Design review of the part built by this model. Coordinates are the model's own, in mm. Face numbers are marked on the shaded views. A direction names the side the tool comes from. Round coordinates to 2 decimals unless told otherwise and drop trailing zeros. Write each loop counter-clockwise with the first axis right and the second up, starting at its lowest first coordinate (ties: lowest second). Pieces come first, ordered by that corner, then holes.
from build123d import *

# Parameters (mm, degrees)
BOSS_EXTRUDE1_DEPTH   = 7.5
CUT_EXTRUDE1_REACH    = 84.706
SKETCH2_R             = 3.4
SKETCH3_R             = 14.05
SKETCH3_R_2           = 10.05
CUT_EXTRUDE2_DEPTH    = 15
FILLET1_R             = 5
M5_TAPPED_HOLE1_D     = 4.2
BODY_MOVE_COPY1_ANGLE = 180


with BuildPart() as part:
    # Sketch1 → Boss-Extrude1 (new, symmetric)
    with BuildSketch(Plane.XY):
        Polygon((40, 0), (-40, 0), (-40, 10), (-25, 10), (-25, 25), (-40, 25), (-40, 72), (40, 72), (40, 25), (25, 25), (25, 10), (40, 10), align=None)
    extrude(amount=BOSS_EXTRUDE1_DEPTH, both=True)

    # Sketch2 → Cut-Extrude1 (cut, up to next)
    with BuildSketch(Plane.XZ, mode=Mode.PRIVATE) as cut_extrude1_sk1:
        with Locations(Location((-35, 0, 0), (0, 0, 270))):
            Circle(SKETCH2_R)
    cut_extrude1_tool1 = extrude(cut_extrude1_sk1.sketch, amount=-CUT_EXTRUDE1_REACH, mode=Mode.PRIVATE) & part.part
    # Sketch2 → Cut-Extrude1 (cut, up to next)
    with BuildSketch(Plane.XZ, mode=Mode.PRIVATE) as cut_extrude1_sk2:
        with Locations(Location((35, 0, 0), (0, 0, 270))):
            Circle(SKETCH2_R)
    cut_extrude1_tool2 = extrude(cut_extrude1_sk2.sketch, amount=-CUT_EXTRUDE1_REACH, mode=Mode.PRIVATE) & part.part
    add(cut_extrude1_tool1.solids().sort_by_distance((-35, 0, 0))[0], mode=Mode.SUBTRACT)
    add(cut_extrude1_tool2.solids().sort_by_distance((35, 0, 0))[0], mode=Mode.SUBTRACT)

    # Sketch3 → Cut-Extrude2 (cut)
    with BuildSketch(Plane.XY.offset(7.5)):
        with Locations((-20, 52)):
            Circle(SKETCH3_R)
        with Locations((20, 52)):
            Circle(SKETCH3_R_2)
    extrude(amount=-CUT_EXTRUDE2_DEPTH, mode=Mode.SUBTRACT)

    # Fillet1
    fillet1_edges = [part.edges().sort_by_distance(p)[0] for p in [
        (-25, 10, 0),
        (-25, 25, 0),
        (-40, 25, 0),
        (-40, 72, 0),
        (40, 72, 0),
        (40, 25, 0),
        (25, 25, 0),
        (25, 10, 0),
    ]]
    fillet(fillet1_edges, radius=FILLET1_R)

    # M5 Tapped Hole1 (through all)
    with Locations(Plane(origin=(0, 0, -7.5), x_dir=(-1, 0, 0), z_dir=(0, 0, -1))):
        with Locations((33.435028843, 38.564971157), (6.564971157, 38.564971157), (6.564971157, 65.435028843), (33.435028843, 65.435028843)):
            Hole(M5_TAPPED_HOLE1_D / 2)


with BuildPart() as part_1:
    # Body-Move/Copy1: moved
    add(part.part.rotate(Axis((0, 30, 0), (0, 0, 1)), BODY_MOVE_COPY1_ANGLE))


solid = part_1.part
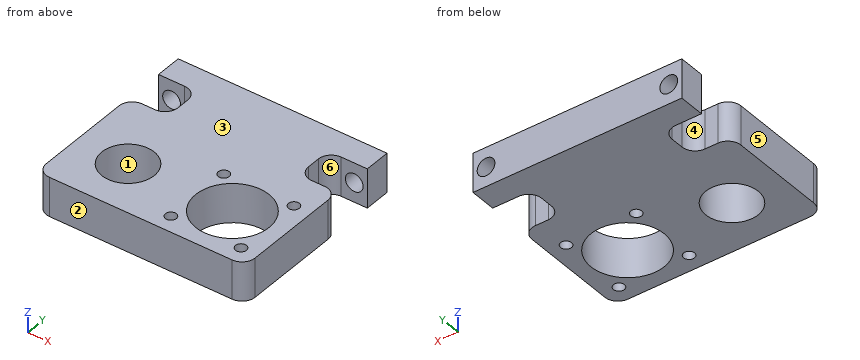
1) For line 1 along X through (y, z) = (8.5, -6.25); line 2 along Y through (x, z) = (20, -2.25); line 3 along Y through (x, z) = (-31.5, 6), list the stretches that pass through material, from the lowest coordinate up.
2) For the marked faces 4, 5 and 6, list the 3-axis set-ups (+Z, -Z, +X, -X, +Y, -Y) from which the entire face can be reached by the end or side of a thin tool; tool diameter is ignored.
3) The part is to be moulded in two halves that separate along Y. For the marked faces 1, 2 and 3, say which applies: pulls with the +Y half, pulls with the -Y half, needs draft (parallel to the pull), parting line crosses it, or undercut.
4) Add section C-C on z = -1.25. Count the separate pieces of the cut face and the enclosed holes in it, and give its area (3 significant figures).
5) Add section D-D on x = 28. State the section outline as (y, z) points, and give its area (3 significant figures).
6) For P1, Ø6, axis at x = -35, z = 0, coming from the +Y side; P2, Ø5.5, axis at y = 43, z = 0.5, coming from the -X side; P3, Ø1, axis at y = 37.5, z = 1.5, coming from the -X side, all flat-tipped, find the tip position at first contact; note any pin that passes through.
7) Add section A-A on x = -20. State the section outline as (y, z) points, and give its area (4 significant figures).
8) Add section B-B on y = 13. State the section outline as (x, z) points, and give its area (3 significant figures).
Computed:
1. line 1: x = -40 to -30.04, -9.96 to 5.96, 34.04 to 40
1. line 2: y = -12 to -6.05, 22.05 to 60
1. line 3: y = -12 to 35, 50 to 60
2. face 4: +Z, -Z, -X
2. face 5: +Z, -Z, -X, +Y, -Y
2. face 6: +Z, -Z, +X
3. face 1: undercut
3. face 2: pulls with the -Y half
3. face 3: needs draft
4. separate pieces: 3
4. enclosed holes: 6
4. area: 4,190 mm2
5. outline: (-12, -7.5) - (-3.55, -7.5) - (-3.55, 7.5) - (-12, 7.5) - close; (19.55, -7.5) - (35.42, -7.5) - (35.42, 7.5) - (19.55, 7.5) - close; (49.58, -7.5) - (60, -7.5) - (60, 7.5) - (49.58, 7.5) - close
5. area: 521 mm2
6. P1: stops at y = 35
6. P2: stops at x = -25.06
6. P3: stops at x = -26
7. outline: (-12, -7.5) - (-2.05, -7.5) - (-2.05, 7.5) - (-12, 7.5) - close; (18.05, -7.5) - (60, -7.5) - (60, 7.5) - (18.05, 7.5) - close
7. area: 778.5 mm2
8. outline: (-40, -7.5) - (-28.72, -7.5) - (-28.72, 7.5) - (-40, 7.5) - close; (-11.28, -7.5) - (6.87, -7.5) - (6.87, 7.5) - (-11.28, 7.5) - close; (33.13, -7.5) - (40, -7.5) - (40, 7.5) - (33.13, 7.5) - close
8. area: 545 mm2
